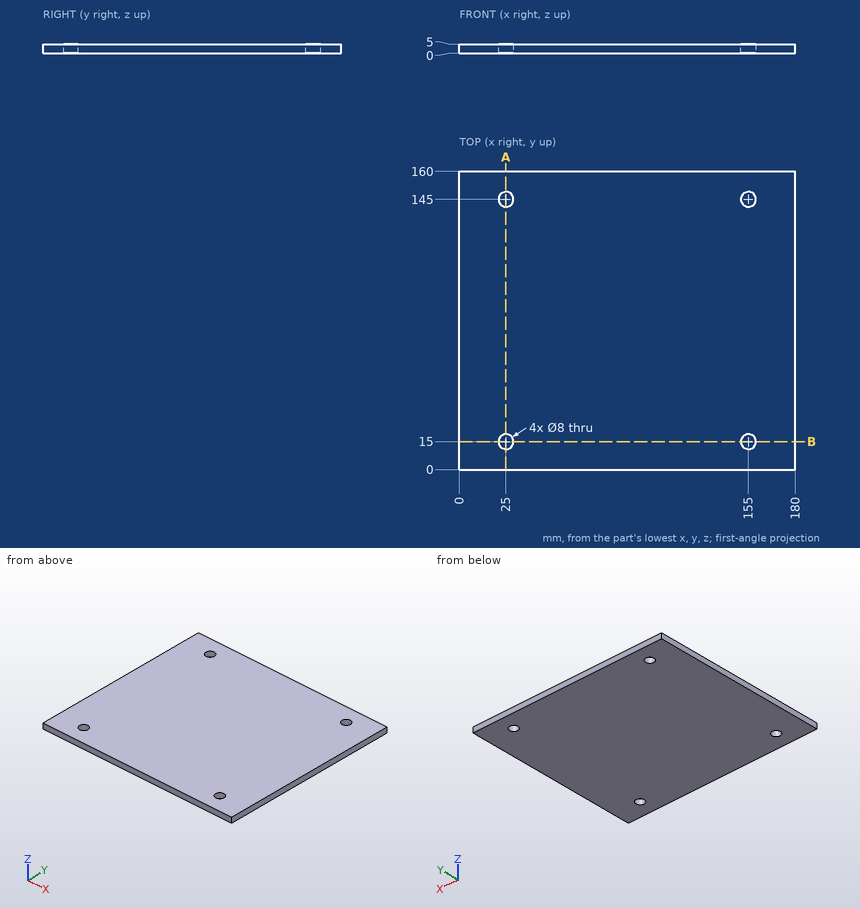
Could you check a few things on this drawing? It's one solid part, dimensions in mm from its lowest x, y, z. Coordinates: 2 decimals unless noted, no trailing zeros. Write each loop counter-clockwise with the first axis right and the second up, starting at its lowest first coordinate (ties: lowest second). Pieces come first, ordered by that corner, then holes. Notation, with made-up numbers: (64.5, -25.75) - (88.5, -25.75) arc R18 ccw to (88.5, -9.75) - close; hole circle Ø8 at (-38, 64.25). An arc over 180 degrees is marked (long way). Return JSON: item names as keys, results as strings. Group by question number.
Item 1: I'm going to push a flat-ended pin straight in: pin 1 Ø5 at (x, y) = (25, 145) entering from -Z. Where does the tip first touch, or does it pass through?
Item 2: If we section it at B-B (y = 15): Write out the boundary of the cut face in (x, z), then the cut area to 3 significant figures.
Item 3: If we section it at A-A (x = 25): Write out the boundary of the cut face in (y, z), then the cut area to 3 significant figures.
Item 4: Please list where these lines run through material, in increasing order: probe 1 along X at (y, z) = (145, 2.35); probe 2 along Y at (x, z) = (155, 2.05).
Return value:
{
 "1": {"pin 1": "passes through"},
 "2": {"outline": "(0, 0) - (21, 0) - (21, 5) - (0, 5) - close; (29, 0) - (151, 0) - (151, 5) - (29, 5) - close; (159, 0) - (180, 0) - (180, 5) - (159, 5) - close", "area": "820 mm^2"},
 "3": {"outline": "(0, 0) - (11, 0) - (11, 5) - (0, 5) - close; (19, 0) - (141, 0) - (141, 5) - (19, 5) - close; (149, 0) - (160, 0) - (160, 5) - (149, 5) - close", "area": "720 mm^2"},
 "4": {"probe 1": "x = 0 to 21, 29 to 151, 159 to 180", "probe 2": "y = 0 to 11, 19 to 141, 149 to 160"}
}
